Here's how the part is built. I have some questions about the finished solid (model axes, mm). A direction names the side the tool comes from. Give positions to 0.01 mm unless a question says otherwise; leave off trailing zeros. Loops run counter-clockwise (first coordinate to the right, second up) from the corner with the lowest first, then second, coordinate; pieces in that order, holes last. Notation, with made-up numbers: (78.5, 58.25) -> (133.5, 58.25) arc R20 cw to (133.5, 89.25) -> close; hole circle Ø3 at (15, -34.5). An arc over 180 degrees is marked (long way). Answer in a Markdown table with one row per item. Add a question column.
Item 1: For P1, Ø8, axis at x = 10, y = 32.5, coming from the -Z side; P2, Ø10, axis at x = 28.5, y = 45, coming from the -Z side, each with a flat end and sliding along its axis, tell me the tip position at first contact or that it passes through.
Item 2: If we section it at D-D (z = -25.5): Write out the boundary of the cut face in (x, y), then the cut area to 3 significant figures.
Item 3: If we section it at B-B (y = 32.5): Write out the boundary of the cut face in (x, z), then the cut area to 3 significant figures.
Item 4: If I drill on line 1 (Y direction, x = 50, z = -3.2); line 2 (X direction, y = 32, z = -3); line 3 (Z direction, x = 5.5, y = 23.5), over which ranges is the centre line in solid material (lowest first)?
Item 5: If we section it at C-C (x = 30): Write out the boundary of the cut face in (y, z).
Item 6: We'd pull the mould along Y, two halves only. Please class faces 1 (the face through (60, 30, -4)), 2 (the face through (46.86, 31.2, -2.43)), 3 (the face through (30, 0, -20)), 4 (the face through (29.6, 60.2, -39)): released by +Y, released by -Y, zero draft, split by the parting line, or undercut.
Item 7: If we section it at A-A (x = 50): Write out the boundary of the cut face in (y, z), then the cut area to 3 significant figures.
Item 8: Which directions (+Z, -Z, +X, -X, +Y, -Y) give clear straight access to the entire face, cutting with the end or side of a thin tool? Please do faces 5 (the face through (29.58, 4.74, -39.05)), 6 (the face through (10.74, 29.18, -2.43)).
```python
from build123d import *

# Parameters (mm, degrees)
MEMBER_C_6_5_1_DEPTH = 60
HOLE_WIZARD_M8_1_D   = 6.8


with BuildPart() as part:
    # Sketch11 → Member C _ 6.5_1 (new body)
    with BuildSketch(Plane(origin=(0, 0, 0), x_dir=(0, 0, -1), z_dir=(1, 0, 0))):
        with BuildLine():
            Line((40, 65), (0, 65))
            Line((0, 65), (0, 0))
            Line((0, 0), (40, 0))
            Line((40, 0), (40, 2.228630091))
            ThreePointArc((40, 2.228630091), (39.023950337, 4.771326395), (36.59720816, 6.007813293))
            Line((36.59720816, 6.007813293), (11.516036525, 8.643950658))
            ThreePointArc((11.516036525, 8.643950658), (6.726413809, 11.084385325), (4.8, 16.102864873))
            Line((4.8, 16.102864873), (4.8, 48.897135127))
            ThreePointArc((4.8, 48.897135127), (6.726413809, 53.915614675), (11.516036525, 56.356049342))
            Line((11.516036525, 56.356049342), (36.59720816, 58.992186707))
            ThreePointArc((36.59720816, 58.992186707), (39.023950337, 60.228673605), (40, 62.771369909))
            Line((40, 62.771369909), (40, 65))
        make_face()
    extrude(amount=MEMBER_C_6_5_1_DEPTH)

    # M8 螺纹孔1 (through all)
    with Locations(Plane(origin=(10, 32.5, 0), x_dir=(1, 0, 0), z_dir=(0, 0, 1))):
        with Locations((0, 0), (40, 0)):
            Hole(HOLE_WIZARD_M8_1_D / 2)


solid = part.part
```
Recorded:
| question | item | result |
|---|---|---|
| 1 | P1 | stops at z = -4.8 |
| 1 | P2 | stops at z = -4.88 |
| 2 | outline | (0, 0) -> (60, 0) -> (60, 7.17) -> (0, 7.17) -> close; (0, 57.83) -> (60, 57.83) -> (60, 65) -> (0, 65) -> close |
| 2 | area | 861 mm^2 |
| 3 | outline | (0, -4.8) -> (6.6, -4.8) -> (6.6, 0) -> (0, 0) -> close; (13.4, -4.8) -> (46.6, -4.8) -> (46.6, 0) -> (13.4, 0) -> close; (53.4, -4.8) -> (60, -4.8) -> (60, 0) -> (53.4, 0) -> close |
| 3 | area | 223 mm^2 |
| 4 | line 1 | y = 0 to 29.1, 35.9 to 65 |
| 4 | line 2 | x = 0 to 6.64, 13.36 to 46.64, 53.36 to 60 |
| 4 | line 3 | z = -4.8 to 0 |
| 5 | outline | (0, -40) -> (2.23, -40) arc R3.8 ccw to (6.01, -36.6) -> (8.64, -11.52) arc R7.5 cw to (16.1, -4.8) -> (48.9, -4.8) arc R7.5 cw to (56.36, -11.52) -> (58.99, -36.6) arc R3.8 ccw to (62.77, -40) -> (65, -40) -> (65, 0) -> (0, 0) -> close |
| 6 | face 1 | zero draft |
| 6 | face 2 | undercut |
| 6 | face 3 | released by -Y |
| 6 | face 4 | undercut |
| 7 | outline | (0, -40) -> (2.23, -40) arc R3.8 ccw to (6.01, -36.6) -> (8.64, -11.52) arc R7.5 cw to (16.1, -4.8) -> (29.1, -4.8) -> (29.1, 0) -> (0, 0) -> close; (35.9, -4.8) -> (48.9, -4.8) arc R7.5 cw to (56.36, -11.52) -> (58.99, -36.6) arc R3.8 ccw to (62.77, -40) -> (65, -40) -> (65, 0) -> (35.9, 0) -> close |
| 7 | area | 821 mm^2 |
| 8 | face 5 | -Z, +X, -X |
| 8 | face 6 | +Z, -Z |
